from build123d import *

# Parameters (mm, degrees)
SKETCH1_R          = 1.25
BASE_EXTRUDE_DEPTH = 1.75


with BuildPart() as part:
    # Sketch1 → Base-Extrude (new body)
    with BuildSketch(Plane.XY):
        with BuildLine():
            Line((-6.879499755, -16.608581611), (-8.323364654, -20.094379832))
            ThreePointArc((-8.323364654, -20.094379832), (0, 21.75), (8.323364654, -20.094379832))
            Line((8.323364654, -20.094379832), (6.879499755, -16.608581611))
            ThreePointArc((6.879499755, -16.608581611), (7.876948304, -13.523963446), (11.081029231, -14.017560694))
            ThreePointArc((11.081029231, -14.017560694), (12.16700015, -14.536168573), (13.28459359, -14.08976979))
            ThreePointArc((13.28459359, -14.08976979), (0, 17.65), (-13.28459359, -14.08976979))
            ThreePointArc((-13.28459359, -14.08976979), (-12.16700015, -14.536168573), (-11.081029231, -14.017560694))
            ThreePointArc((-11.081029231, -14.017560694), (-7.876948304, -13.523963446), (-6.879499755, -16.608581611))
        make_face()
        with Locations((-9.363022706, -16.071521577)):
            Circle(SKETCH1_R, mode=Mode.SUBTRACT)
        with Locations(Location((9.363022706, -16.071521577, 0), (0, 0, 180))):
            Circle(SKETCH1_R, mode=Mode.SUBTRACT)
    extrude(amount=BASE_EXTRUDE_DEPTH)


solid = part.part
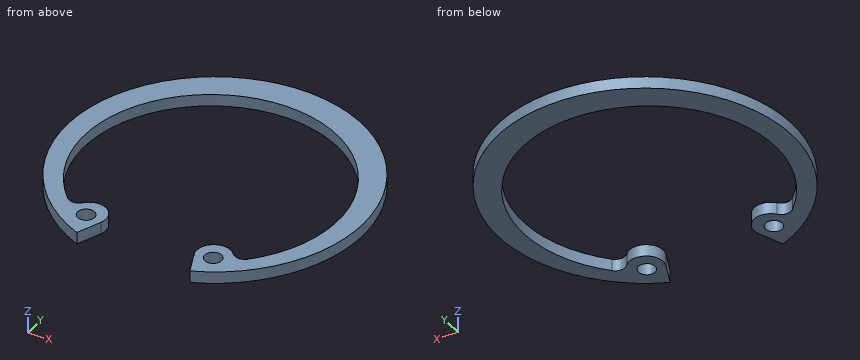
Build history of the part. All positions in model axes, mm. Round coordinates to 2 decimals unless told otherwise and drop trailing zeros. Order: outer loops, then holes, each group sorted by start corner. A loop starts at its lowest first (then second) coordinate and runs counter-clockwise, first axis right, second up. Notation, with made-up numbers: M 75.5,16 L 103.5,16 A14 cw 103.5,27 Z; hole C -29.5,84.25 d5. An arc over 180 degrees is marked long. Use CSV: the item, a comma, the result in double quotes. Start each with the question number.
(1) Cut at D-D on y = 8.5. List the corners of the cut face in (x, z).
(2) Flat gauge pin, fed straight in: P1, Ø4, axis at x = -14, y = -9.5, coming from the +Z side. Where does the tip first touch, or does it go through?
(3) Cut at B-B on y = -7.5. List the corners of the cut face in (x, z).
(4) Drill centre lines: probe 1 along X at (y, z) = (-17.5, 0.9); probe 2 along X at (y, z) = (6, 0.15); probe 3 along Y at (x, z) = (8, 1.05). Where is each one in solid material? Low to high.
(5) Cut at C-C on z = 1.05. List the corners of the cut face in (x, y), then the cut area to 3 significant figures.
(6) Cut at A-A on x = 9.5. List the corners of the cut face in (y, z).
Findings:
1,outline,"M -20.02,0 L -16.05,0 L -16.05,1.75 L -20.02,1.75 Z; M 16.05,0 L 20.02,0 L 20.02,1.75 L 16.05,1.75 Z"
2,P1,"passes through"
3,outline,"M -20.42,0 L -17.48,0 L -17.48,1.75 L -20.42,1.75 Z; M 17.48,0 L 20.42,0 L 20.42,1.75 L 17.48,1.75 Z"
4,probe 1,"x = -12.92 to -7.25, 7.25 to 12.92"
4,probe 2,"x = -20.91 to -17.29, 17.29 to 20.91"
4,probe 3,"y = -19.31 to -13.45, 15.85 to 20.23"
5,outline,"M -13.28,-14.09 A18.65 cw long 13.28,-14.09 A1.5 cw 11.08,-14.02 A2.5 ccw 6.88,-16.61 L 8.32,-20.09 A21.75 ccw long -8.32,-20.09 L -6.88,-16.61 A2.5 ccw -11.08,-14.02 A1.5 cw Z; hole C -9.36,-16.07 d2.5; hole C 9.36,-16.07 d2.5"
5,area,"383 mm^2"
6,outline,"M -19.57,0 L -17.31,0 L -17.31,1.75 L -19.57,1.75 Z; M -14.83,0 L -13.17,0 L -13.17,1.75 L -14.83,1.75 Z; M 15.05,0 L 19.57,0 L 19.57,1.75 L 15.05,1.75 Z"
